Input: part model. Units: mm. Frame: model coordinates. A direction names the side the tool comes from. Round coordinates to 2 decimals unless told otherwise and drop trailing zeros. Write each loop counter-clockwise with the first axis right and the second up, starting at its lowest first coordinate (ties: lowest second). Pieces come first, ordered by that corner, then holes. Notation, with made-up numbers: (75.25, -18.5) -> (94.25, -18.5) arc R21 ccw to (94.25, -6.5) -> close; hole circle Ø5 at (4.25, 13.5). An arc over 180 degrees is marked (long way). Write item = value, one per line.
```python
from build123d import *

# Parameters (mm, degrees)
EXTRUDE_1_DEPTH          = 35
CHAMFER_1_SIZE           = 12
CUT_EXTRUDE_1_DEPTH      = 976.679250574
CUT_EXTRUDE_1_DEPTH_BACK = 976.679250574
SKETCH_2_R               = 11


with BuildPart() as part:
    # 草图1 → 凸台-拉伸1 (new body)
    with BuildSketch(Plane.XY):
        Polygon((0, 0), (0, -485), (-330, -485), (-330, -745), (-80, -745), (-80, -865), (-450, -865), (-450, -365), (-100, -365), (-100, 0), align=None)
    extrude(amount=EXTRUDE_1_DEPTH)

    # 倒角1
    chamfer_1_edges = [part.edges().sort_by_distance(p)[0] for p in [
        (-100, 0, 17.5),
        (-450, -865, 17.5),
        (-450, -365, 17.5),
    ]]
    chamfer(chamfer_1_edges, length=CHAMFER_1_SIZE)

    # 草图2 → 切除-拉伸1 (cut, two sides: drawn at the far end of the back side and taken through both)
    with BuildSketch(Plane.XY.offset(35).offset(-CUT_EXTRUDE_1_DEPTH_BACK)):
        with Locations((-60, -40)):
            Circle(SKETCH_2_R)
        with Locations((-60, -170)):
            Circle(SKETCH_2_R)
        with Locations((-60, -300)):
            Circle(SKETCH_2_R)
        with Locations((-60, -405)):
            Circle(SKETCH_2_R)
        with Locations((-240, -405)):
            Circle(SKETCH_2_R)
        with Locations((-410, -405)):
            Circle(SKETCH_2_R)
        with Locations((-410, -545)):
            Circle(SKETCH_2_R)
        with Locations((-410, -685)):
            Circle(SKETCH_2_R)
        with Locations((-410, -825)):
            Circle(SKETCH_2_R)
        with Locations((-240, -825)):
            Circle(SKETCH_2_R)
    extrude(amount=CUT_EXTRUDE_1_DEPTH + CUT_EXTRUDE_1_DEPTH_BACK, mode=Mode.SUBTRACT)


solid = part.part
```
1) Line query: L1, parallel to Y at x = -60, z = 19.5; L2, parallel to X at y = -405, z = 26; L3, parallel to X at y = -825, z = 9. Output: solid intervals per line, ascending. Write a range as from..to.
Solutions:
L1 = -485..-416, -394..-311, -289..-181, -159..-51, -29..0
L2 = -450..-421, -399..-251, -229..-71, -49..0
L3 = -450..-421, -399..-251, -229..-80
2) Draft query along X for faces 4 (the face through (-222, -426, 35)), 5 (the face through (-330, -613, 17)), 6 (the face through (-100, -191, 17)), 7 (the face through (-412.38, -835.74, 17.25)). Return one class per face: +X half, -X half, draft (parallel to the pull), parting line (faces both ways), or undercut.
Solutions:
face_4 = draft
face_5 = +X half
face_6 = -X half
face_7 = undercut
3) Cut plane D-D (y = -170). Return the cut outline in (x, z).
Solutions:
outline = (-100, 0) -> (-71, 0) -> (-71, 35) -> (-100, 35) -> close; (-49, 0) -> (0, 0) -> (0, 35) -> (-49, 35) -> close
4) Cut plane C-C (z = 12.5). Count the separate pieces of the cut face and the enclosed holes in it, and give its area (3 significant figures).
Solutions:
separate_pieces = 1
enclosed_holes = 10
area = 162,000 mm^2
5) Cut plane A-A (y = -825). Return the cut outline in (x, z), and give its area (3 significant figures).
Solutions:
outline = (-450, 0) -> (-421, 0) -> (-421, 35) -> (-450, 35) -> close; (-399, 0) -> (-251, 0) -> (-251, 35) -> (-399, 35) -> close; (-229, 0) -> (-80, 0) -> (-80, 35) -> (-229, 35) -> close
area = 11,400 mm^2
6) Cut plane B-B (x = -240). Return the cut outline in (y, z), and give its area (3 significant figures).
Solutions:
outline = (-865, 0) -> (-836, 0) -> (-836, 35) -> (-865, 35) -> close; (-814, 0) -> (-745, 0) -> (-745, 35) -> (-814, 35) -> close; (-485, 0) -> (-416, 0) -> (-416, 35) -> (-485, 35) -> close; (-394, 0) -> (-365, 0) -> (-365, 35) -> (-394, 35) -> close
area = 6,860 mm^2
7) First-contact query: P1, Ø17.5, axis at y = -811.5, z = 9.5, coming from the +X side; P2, Ø2, axis at y = -494.5, z = 8.5, coming from the +X side; P3, Ø12, axis at y = -268, z = 14, coming from the -X side. Flat tips, straight axial feed; report the tip coordinate or a pass-through.
Solutions:
P1 = -80
P2 = -330
P3 = -100
8) Access query for faces 1 (the face through (-207, -745, 17)), 2 (the face through (-450, -618, 17)), 3 (the face through (-271, -365, 17)). Directions: +Z, -Z, +X, -X, +Y, -Y. A direction counts if a zero-diameter tool reaches every point of the face in a straight line with its end or side. Return the directions, or none.
Solutions:
face_1 = +Z, -Z, +X
face_2 = +Z, -Z, -X, +Y, -Y
face_3 = +Z, -Z, -X, +Y
